For this review, take the finished solid that the model builds, in its own axes (mm). A direction names the side the tool comes from. Give positions to 0.01 mm unless a question says otherwise; leave off trailing zeros. Write each loop counter-clockwise with the first axis right and the second up, starting at its lowest first coordinate (ties: lowest second). Pieces come first, ordered by that corner, then holes.
1) Machinability: for faces 5 (the face through (45, 109, -66)), 6 (the face through (39.912, 212, -64)), 7 (the face through (-51, 95, -66)), 8 (the face through (-70, 159, -6)), which of the approach directions +Z, -Z, +X, -X, +Y, -Y give a long, thin tool a straight path to every point of the face, cutting with its end or side? Answer none if there is none.
2) We need section C-C on x = 9.5. Give the boundary of the cut face in (y, z).
3) We need section B-B on y = 102.5. Give the boundary of the cut face in (x, z), and give its area (3 significant figures).
4) Draft analysis for pull direction Y (two halves, no side actions). For faces 1 (the face through (-64, 90, -64)), 2 (the face through (-65, 159, -19)), 3 (the face through (-11, 95, -19)), 4 (the face through (45, 159, -19)), state which applies: pulls with the +Y half, pulls with the -Y half, needs draft (parallel to the pull), parting line crosses it, or undercut.
5) Wall thickness on line 1 along Y through (x, z) = (-61.5, -21.5); line 2 along Y through (x, z) = (-45, -12.5); line 3 along X through (y, z) = (123, -114.5): over which ranges is each line inside the solid? List them lowest first.
6) We need section D-D on z = -56.5. Give the boundary of the cut face in (x, y), and give its area (3 significant figures).
7) We need section A-A on y = 156. Give the boundary of the cut face in (x, z).
from build123d import *

# Parameters (mm, degrees)
SKETCH1_W           = 119.911519959
SKETCH1_H           = 140
SKETCH1_W_2         = 99.911519959
SKETCH1_H_2         = 120
BOSS_EXTRUDE1_DEPTH = 130
SKETCH2_W           = 81.911519959
SKETCH2_H           = 92
CUT_EXTRUDE1_DEPTH  = 258
SKETCH3_W           = 92
SKETCH3_H           = 102
CUT_EXTRUDE2_DEPTH  = 258


with BuildPart() as part:
    # Sketch1 → Boss-Extrude1 (new body)
    with BuildSketch(Plane.XY):
        with Locations((-10.04424002, 160)):
            Rectangle(SKETCH1_W, SKETCH1_H)
        with Locations((-10.044240021, 160)):
            Rectangle(SKETCH1_W_2, SKETCH1_H_2, mode=Mode.SUBTRACT)
    extrude(amount=-BOSS_EXTRUDE1_DEPTH)

    # Sketch2 → Cut-Extrude1 (cut)
    with BuildSketch(Plane.XZ.offset(-90)):
        with Locations((-10.04424002, -65)):
            Rectangle(SKETCH2_W, SKETCH2_H)
    extrude(amount=-CUT_EXTRUDE1_DEPTH, mode=Mode.SUBTRACT)

    # Sketch3 → Cut-Extrude2 (cut)
    with BuildSketch(Plane.ZY.offset(70)):
        with Locations((-65, 160)):
            Rectangle(SKETCH3_W, SKETCH3_H)
    extrude(amount=-CUT_EXTRUDE2_DEPTH, mode=Mode.SUBTRACT)


solid = part.part
Results list:
1. face 5: +X, -X
1. face 6: +Z, -Z
1. face 7: +Y, -Y
1. face 8: +Z, -Z, -X, +Y, -Y
2. outline: (90, -130) - (100, -130) - (100, -111) - (90, -111) - close; (90, -19) - (100, -19) - (100, 0) - (90, 0) - close; (220, -130) - (230, -130) - (230, -111) - (220, -111) - close; (220, -19) - (230, -19) - (230, 0) - (220, 0) - close
3. outline: (-70, -130) - (-60, -130) - (-60, 0) - (-70, 0) - close; (39.91, -130) - (49.91, -130) - (49.91, 0) - (39.91, 0) - close
3. area: 2,600 mm2
4. face 1: pulls with the -Y half
4. face 2: undercut
4. face 3: needs draft
4. face 4: undercut
5. line 1: y = 90 to 109, 211 to 230
5. line 2: y = 90 to 100, 220 to 230
5. line 3: x = -70 to -60, 39.91 to 49.91
6. outline: (-70, 90) - (-51, 90) - (-51, 100) - (-60, 100) - (-60, 109) - (-70, 109) - close; (-70, 211) - (-60, 211) - (-60, 220) - (-51, 220) - (-51, 230) - (-70, 230) - close; (30.91, 90) - (49.91, 90) - (49.91, 109) - (39.91, 109) - (39.91, 100) - (30.91, 100) - close; (30.91, 220) - (39.91, 220) - (39.91, 211) - (49.91, 211) - (49.91, 230) - (30.91, 230) - close
6. area: 1,120 mm2
7. outline: (-70, -130) - (-60, -130) - (-60, -111) - (-70, -111) - close; (-70, -19) - (-60, -19) - (-60, 0) - (-70, 0) - close; (39.91, -130) - (49.91, -130) - (49.91, -111) - (39.91, -111) - close; (39.91, -19) - (49.91, -19) - (49.91, 0) - (39.91, 0) - close
